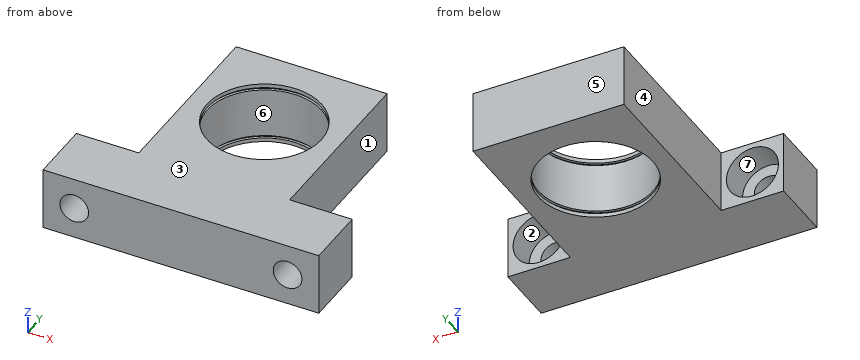
from build123d import *

# Parameters (mm, degrees)
SKETCH_1_R          = 11
EXTRUDE_1_DEPTH     = 12
SKETCH_2_R          = 2.75
CUT_EXTRUDE_1_DEPTH = 53.135542299
SKETCH_3_R          = 5
CUT_EXTRUDE_2_DEPTH = 5.8
SKETCH_4_R          = 11.5
CUT_EXTRUDE_3_DEPTH = 0.25
SKETCH_5_R          = 11.5
CUT_EXTRUDE_4_DEPTH = 0.25


with BuildPart() as part:
    # 草图1 → 凸台-拉伸1 (new body)
    with BuildSketch(Plane.XY):
        Polygon((-16.269702277, -16.03765324), (36.730297723, -16.03765324), (36.730297723, -4.03765324), (24.730297723, -4.03765324), (24.730297723, 30.96234676), (-4.269702277, 30.96234676), (-4.269702277, -4.03765324), (-16.269702277, -4.03765324), align=None)
        with Locations((10.230297723, 13.96234676)):
            Circle(SKETCH_1_R, mode=Mode.SUBTRACT)
    extrude(amount=EXTRUDE_1_DEPTH)

    # 草图2 → 切除-拉伸1 (cut, through all)
    with BuildSketch(Plane(origin=(0, -4.03765324, 0), x_dir=(1, 0, 0), z_dir=(0, 1, 0))):
        with Locations(Location((-10.269702277, -6, 0), (0, 0, 180))):
            Circle(SKETCH_2_R)
        with Locations(Location((30.730297723, -6, 0), (0, 0, 180))):
            Circle(SKETCH_2_R)
    extrude(amount=-CUT_EXTRUDE_1_DEPTH, mode=Mode.SUBTRACT)

    # 草图3 → 切除-拉伸2 (cut)
    with BuildSketch(Plane(origin=(0, -4.03765324, 0), x_dir=(1, 0, 0), z_dir=(0, 1, 0))):
        with Locations(Location((-10.269702277, -6, 0), (0, 0, 180))):
            Circle(SKETCH_3_R)
        with Locations(Location((30.730297723, -6, 0), (0, 0, 180))):
            Circle(SKETCH_3_R)
    extrude(amount=-CUT_EXTRUDE_2_DEPTH, mode=Mode.SUBTRACT)

    # 草图4 → 切除-拉伸3 (cut, symmetric)
    with BuildSketch(Plane.XY.offset(11)):
        with Locations((10.230297723, 13.96234676)):
            Circle(SKETCH_4_R)
    extrude(amount=CUT_EXTRUDE_3_DEPTH, both=True, mode=Mode.SUBTRACT)

    # 草图5 → 切除-拉伸4 (cut, symmetric)
    with BuildSketch(Plane(origin=(0, 0, 1), x_dir=(-1, 0, 0), z_dir=(0, 0, -1))):
        with Locations(Location((-10.230297723, 13.96234676, 0), (0, 0, 180))):
            Circle(SKETCH_5_R)
    extrude(amount=CUT_EXTRUDE_4_DEPTH, both=True, mode=Mode.SUBTRACT)


solid = part.part
Verification items for the finished model (mm, model axes). Face numbers are marked on the shaded views. A direction names the side the tool comes from. Coordinates: 2 decimals unless noted, no trailing zeros. Order: outer loops, then holes, each group sorted by start corner. A loop starts at its lowest first (then second) coordinate and runs counter-clockwise, first axis right, second up.
Item 1: Section check B-B, the plane x = 10. Enter the section's corners in (y, z), then the cut area to 3 significant figures.
Filled in:
outline: (-16.04, 0) - (2.96, 0) - (2.96, 0.75) - (2.46, 0.75) - (2.46, 1.25) - (2.96, 1.25) - (2.96, 10.75) - (2.46, 10.75) - (2.46, 11.25) - (2.96, 11.25) - (2.96, 12) - (-16.04, 12) - close; (24.96, 0) - (30.96, 0) - (30.96, 12) - (24.96, 12) - (24.96, 11.25) - (25.46, 11.25) - (25.46, 10.75) - (24.96, 10.75) - (24.96, 1.25) - (25.46, 1.25) - (25.46, 0.75) - (24.96, 0.75) - close
area: 299 mm2
Item 2: Material ranges on L1, parallel to X at y = 28, z = 6; L2, parallel to X at y = 18, z = 5.5; L3, parallel to Y at x = 1, z = 7.25, recorded low to high.
Filled in:
L1: x = -4.27 to 24.73
L2: x = -4.27 to 0, 20.46 to 24.73
L3: y = -16.04 to 7.98, 19.95 to 30.96
Item 3: Section check A-A, the plane z = 8. Enter the section's corners in (x, y), then the cut area to 3 significant figures.
Filled in:
outline: (-16.27, -16.04) - (-12.16, -16.04) - (-12.16, -9.84) - (-14.85, -9.84) - (-14.85, -4.04) - (-16.27, -4.04) - close; (-8.38, -16.04) - (28.84, -16.04) - (28.84, -9.84) - (26.15, -9.84) - (26.15, -4.04) - (24.73, -4.04) - (24.73, 30.96) - (-4.27, 30.96) - (-4.27, -4.04) - (-5.69, -4.04) - (-5.69, -9.84) - (-8.38, -9.84) - close; (32.62, -16.04) - (36.73, -16.04) - (36.73, -4.04) - (35.31, -4.04) - (35.31, -9.84) - (32.62, -9.84) - close; hole circle Ø22 at (10.23, 13.96)
area: 1,120 mm2
Item 4: Release check for a two-part mould opening along Y. For the marked faces 5, 6 and 7 record: +Y half, -Y half, draft (parallel to the pull), parting line (faces both ways), or undercut.
Filled in:
face 5: +Y half
face 6: undercut
face 7: draft
Item 5: Section check C-C, the plane y = 22.5. Enter the section's corners in (x, z), then the cut area to 3 significant figures.
Filled in:
outline: (-4.27, 0) - (3.29, 0) - (3.29, 0.75) - (2.53, 0.75) - (2.53, 1.25) - (3.29, 1.25) - (3.29, 10.75) - (2.53, 10.75) - (2.53, 11.25) - (3.29, 11.25) - (3.29, 12) - (-4.27, 12) - close; (17.17, 0) - (24.73, 0) - (24.73, 12) - (17.17, 12) - (17.17, 11.25) - (17.93, 11.25) - (17.93, 10.75) - (17.17, 10.75) - (17.17, 1.25) - (17.93, 1.25) - (17.93, 0.75) - (17.17, 0.75) - close
area: 180 mm2
Item 6: Access from +Z, -Z, +X, -X, +Y, -Y to the whole of each face (thin tool, end or side, straight path). Record for the marked faces 1, 2, 3 and 4.
Filled in:
face 1: +Z, -Z, +X, +Y
face 2: +Y
face 3: +Z, +X, -X, +Y, -Y
face 4: +Z, -Z, -X, +Y
Item 7: Depth check by flat-ended pin: pin 1 (2 mm diameter, centred on y = 24.5, z = 1.5, fed in from +X); pin 2 (5 mm diameter, centred on x = -12, z = 5, fed in from +Y); pin 3 (5 mm diameter, centred on y = 16, z = 9, fed in from -X). Enter the tip coordinate at first touch or a pass-through.
Filled in:
pin 1: stops at x = 24.73
pin 2: stops at y = -9.84
pin 3: stops at x = -4.27
Item 8: Section check D-D, the plane z = 2.5. Enter the section's corners in (x, y).
Filled in:
outline: (-16.27, -16.04) - (36.73, -16.04) - (36.73, -4.04) - (34.3, -4.04) - (34.3, -9.84) - (27.16, -9.84) - (27.16, -4.04) - (24.73, -4.04) - (24.73, 30.96) - (-4.27, 30.96) - (-4.27, -4.04) - (-6.7, -4.04) - (-6.7, -9.84) - (-13.84, -9.84) - (-13.84, -4.04) - (-16.27, -4.04) - close; hole circle Ø22 at (10.23, 13.96)
